from build123d import *

# Parameters (mm, degrees)
SKETCH1_W            = 110
SKETCH1_H            = 350
BOSS_EXTRUDE1_DEPTH  = 80
SHELL1_T             = -10
SKETCH2_W            = 20
SKETCH2_H            = 60
BOSS_EXTRUDE2_DEPTH  = 20
SKETCH3_W            = 15
SKETCH3_H            = 50
CUT_EXTRUDE1_DEPTH   = 50
FILLET1_R            = 10
FILLET1_OF_MIRROR1_R = 10
SKETCH4_R            = 15
CUT_EXTRUDE2_DEPTH   = 50


with BuildPart() as part:
    # Sketch1 → Boss-Extrude1 (new body)
    with BuildSketch(Plane.XY):
        with Locations((-119, 670)):
            Rectangle(SKETCH1_W, SKETCH1_H)
    extrude(amount=BOSS_EXTRUDE1_DEPTH)

    # Shell1
    shell1_openings = [part.faces().sort_by_distance(p)[0] for p in [
        (-119, 670, 80),
    ]]
    offset(amount=SHELL1_T, openings=shell1_openings, kind=Kind.INTERSECTION)

    # Sketch2 → Boss-Extrude2 (add)
    with BuildSketch(Plane.ZY.offset(174)):
        with Locations((40, 732.363495956)):
            Rectangle(SKETCH2_W, SKETCH2_H)
        with Locations((40, 571.241967209)):
            Rectangle(SKETCH2_W, SKETCH2_H)
    boss_extrude2 = extrude(amount=BOSS_EXTRUDE2_DEPTH)

    # Sketch3 → Cut-Extrude1 (cut)
    with BuildSketch(Plane.XY.offset(50)):
        Polygon((-179, 596.241967209), (-174, 596.241967209), (-174, 546.241967209), (-179, 546.241967209), (-189, 546.241967209), (-189, 596.241967209), align=None)
        with Locations((-181.5, 732.363495956)):
            Rectangle(SKETCH3_W, SKETCH3_H)
    cut_extrude1 = extrude(amount=-CUT_EXTRUDE1_DEPTH, mode=Mode.SUBTRACT)

    # Fillet1
    fillet1_edges = [part.edges().sort_by_distance(p)[0] for p in [
        (-194, 702.363495956, 40),
        (-194, 762.363495956, 40),
        (-194, 541.241967209, 40),
        (-194, 601.241967209, 40),
        (-189, 546.241967209, 40),
        (-189, 596.241967209, 40),
        (-189, 707.363495956, 40),
        (-189, 757.363495956, 40),
    ]]
    fillet(fillet1_edges, radius=FILLET1_R)

    # Mirror1: Boss-Extrude2, Cut-Extrude1 across plane
    add(boss_extrude2.mirror(Plane(origin=(-119, 0, 0), x_dir=(0, 0, 1), z_dir=(1, 0, 0))))
    add(cut_extrude1.mirror(Plane(origin=(-119, 0, 0), x_dir=(0, 0, 1), z_dir=(1, 0, 0))), mode=Mode.SUBTRACT)

    # Fillet1 of Mirror1
    fillet1_of_mirror1_edges = [part.edges().sort_by_distance(p)[0] for p in [
        (-44, 702.363495956, 40),
        (-44, 762.363495956, 40),
        (-44, 541.241967209, 40),
        (-44, 601.241967209, 40),
        (-49, 546.241967209, 40),
        (-49, 596.241967209, 40),
        (-49, 707.363495956, 40),
        (-49, 757.363495956, 40),
    ]]
    fillet(fillet1_of_mirror1_edges, radius=FILLET1_OF_MIRROR1_R)

    # Sketch4 → Cut-Extrude2 (cut)
    with BuildSketch(Plane(origin=(0, 845, 0), x_dir=(1, 0, 0), z_dir=(0, 1, 0))):
        with Locations(Location((-119, -40, 0), (0, 0, 270))):
            Circle(SKETCH4_R)
    extrude(amount=-CUT_EXTRUDE2_DEPTH, mode=Mode.SUBTRACT)


solid = part.part
Geometry: final body of the model. Coordinates: model frame, mm. A direction names the side the tool comes from. Round coordinates to 2 decimals unless told otherwise and drop trailing zeros. Order: outer loops, then holes, each group sorted by start corner. A loop starts at its lowest first (then second) coordinate and runs counter-clockwise, first axis right, second up. Notation, with made-up numbers: (-40, 81.5) - (5, 81.5) arc R15 ccw to (5, 109.5) - close; hole circle Ø5 at (21, -26). An arc over 180 degrees is marked (long way). Write each question's results on one line, items separated by ' | '.
Item 1: Material intervals for line 1 along X through (y, z) = (815.5, 25.5); line 2 along Y through (x, z) = (-88, 51.5); line 3 along X through (y, z) = (586, 42), sorted ascending. Write a range as [from, to].
Completed:
line 1: [-174, -164], [-74, -64] | line 2: [495, 505], [835, 845] | line 3: [-194, -189], [-174, -164], [-74, -64], [-49, -44]
Item 2: Reachability of faces 5 (the cylindrical face through (-51.85, 710.37, 39.86)), 6 (the flat face through (-59, 762.363, 40)), 7 (the flat face through (-47, 571, 30)), 8 (the flat face through (-59, 702.363, 40)), 9 (the flat face through (-120, 672, 10)) from +Z, -Z, +X, -X, +Y, -Y: full face, straight path, thin tool, end or side. Return the list, or none.
Completed:
face 5: +Z, -Z | face 6: +Z, -Z, +X, +Y | face 7: -Z, +X, +Y, -Y | face 8: +Z, -Z, +X | face 9: +Z
Item 3: Section D-D, the plane y = 611. Return the cut outline in (x, z), and give its area (3 significant figures).
Completed:
outline: (-174, 0) - (-64, 0) - (-64, 80) - (-74, 80) - (-74, 10) - (-164, 10) - (-164, 80) - (-174, 80) - close | area: 2,500 mm^2
Item 4: Section C-C, the plane x = -87.5. Return the cut outline in (y, z).
Completed:
outline: (495, 0) - (845, 0) - (845, 80) - (835, 80) - (835, 10) - (505, 10) - (505, 80) - (495, 80) - close
Item 5: First-contact query: pin 1 Ø1 at (y, z) = (766, 40) entering from -X; pin 2 Ø5 at (x, z) = (-180, 37.5) entering from -Y; pin 3 Ø2 at (x, y) = (-176, 614) entering from -Z; pin 4 Ø2 at (x, y) = (-159, 611) entering from -Z. Flat tips, straight axial feed; report the tip coordinate or a pass-through.
Completed:
pin 1: x = -174 | pin 2: y = 541.24 | pin 3: through | pin 4: z = 0
Item 6: Mould query, pull axis X, two halves, no side actions, for faces 1 (the flat face through (-191, 732, 30)), 2 (the flat face through (-189, 732, 40)), 3 (the cylindrical face through (-46.85, 705.37, 40.14)), 4 (the flat face through (-120, 505, 45)). Classes: pulls with the +X half, pulls with the -X half, needs draft (parallel to the pull), parting line crosses it, or undercut.
Completed:
face 1: needs draft | face 2: undercut | face 3: pulls with the +X half | face 4: undercut
Item 7: Section B-B, the plane z = 67. Return the cut outline in (x, y), and give its area (3 significant figures).
Completed:
outline: (-174, 495) - (-64, 495) - (-64, 845) - (-174, 845) - close; hole (-164, 505) - (-74, 505) - (-74, 835) - (-164, 835) - close | area: 8,800 mm^2
Item 8: Section A-A, the plane x = -119. Return the cut outline in (y, z), and give its area (3 significant figures).
Completed:
outline: (495, 0) - (845, 0) - (845, 25) - (835, 25) - (835, 10) - (505, 10) - (505, 80) - (495, 80) - close; (835, 55) - (845, 55) - (845, 80) - (835, 80) - close | area: 4,600 mm^2
